```python
from build123d import *

# Parameters (mm, degrees)
SKETCH_1_R              = 12.5
EXTRUDE_1_DEPTH         = 111
SKETCH_2_R              = 17.5
EXTRUDE_2_DEPTH         = 3
SKETCH_3_R              = 10
EXTRUDE_3_DEPTH         = 8
CUT_EXTRUDE_1_DEPTH     = 4
HOLE_WIZARD_M8_1_D      = 6.8
HOLE_WIZARD_M8_1_DEPTH  = 23.75
HOLE_WIZARD_M8_1_TIP    = 2.042926105
HOLE_WIZARD_M12_1_D     = 10.2
HOLE_WIZARD_M12_1_DEPTH = 30.25
HOLE_WIZARD_M12_1_TIP   = 3.064389157
CHAMFER_1_SIZE          = 0.5


with BuildPart() as part:
    # 草图1 → 凸台-拉伸1 (new body)
    with BuildSketch(Plane.XY):
        Circle(SKETCH_1_R)
    extrude(amount=EXTRUDE_1_DEPTH)

    # 草图2 → 凸台-拉伸2 (add)
    with BuildSketch(Plane.XY.offset(111)):
        Circle(SKETCH_2_R)
    extrude(amount=EXTRUDE_2_DEPTH)

    # 草图3 → 凸台-拉伸3 (add)
    with BuildSketch(Plane.XY.offset(114)):
        Circle(SKETCH_3_R)
    extrude(amount=EXTRUDE_3_DEPTH)

    # 草图4 → 切除-拉伸1 (cut)
    with BuildSketch(Plane(origin=(0, 12.5, 0), x_dir=(1, 0, 0), z_dir=(0, 1, 0))):
        with BuildLine():
            Line((4, -10), (4, -102))
            ThreePointArc((4, -102), (0, -106), (-4, -102))
            Line((-4, -102), (-4, -10))
            ThreePointArc((-4, -10), (0, -6), (4, -10))
        make_face()
    extrude(amount=-CUT_EXTRUDE_1_DEPTH, mode=Mode.SUBTRACT)

    # M8 螺纹孔1
    with Locations(Plane.XY.offset(122)):
        with Locations((0, 0)):
            Hole(HOLE_WIZARD_M8_1_D / 2, depth=HOLE_WIZARD_M8_1_DEPTH)
            with Locations((0, 0, -(HOLE_WIZARD_M8_1_DEPTH + HOLE_WIZARD_M8_1_TIP / 2))):  # 118° drill point
                Cone(0, HOLE_WIZARD_M8_1_D / 2, HOLE_WIZARD_M8_1_TIP, mode=Mode.SUBTRACT)

    # M12 螺纹孔1
    with Locations(Plane(origin=(0, 0, 0), x_dir=(-1, 0, 0), z_dir=(0, 0, -1))):
        with Locations((0, 0)):
            Hole(HOLE_WIZARD_M12_1_D / 2, depth=HOLE_WIZARD_M12_1_DEPTH)
            with Locations((0, 0, -(HOLE_WIZARD_M12_1_DEPTH + HOLE_WIZARD_M12_1_TIP / 2))):  # 118° drill point
                Cone(0, HOLE_WIZARD_M12_1_D / 2, HOLE_WIZARD_M12_1_TIP, mode=Mode.SUBTRACT)

    # 倒角1
    chamfer_1_edges = [part.edges().sort_by_distance(p)[0] for p in [
        (-12.5, 0, 0),
    ]]
    chamfer(chamfer_1_edges, length=CHAMFER_1_SIZE)


solid = part.part
```
Part model, mm, in its own coordinate system. A direction names the side the tool comes from. Round coordinates to 2 decimals unless told otherwise and drop trailing zeros. Order: outer loops, then holes, each group sorted by start corner. A loop starts at its lowest first (then second) coordinate and runs counter-clockwise, first axis right, second up. Notation, with made-up numbers: M 48,7.5 L 91,7.5 A24 ccw 91,21.5 Z; hole C 25.5,-14.75 d9. An arc over 180 degrees is marked long. Answer in a Markdown table with one row per item. Add a question column.
Q1. Wall check: L1, parallel to Y at x = 0, z = 108; L2, parallel to Y at x = 0, z = 15.5; L3, parallel to Z at x = 13, y = 6.5. Give the ranges that are in metal, low to high. Write a range as from..to.
Q2. Cut at A-A on z = 58.5. Give the cut face in (x, y), and give its area (3 significant figures).
Q3. Mould opens along Y. For faces 1 (the face through (8, -11, 111)), 2 (the face through (0.192, -0.865, 32.782)), 3 (the face through (-2.17, -9.76, 117.94)) say: +Y half, -Y half, draft (parallel to the pull), parting line (faces both ways), or undercut.
Q4. Pin check, flat tips, straight feed: pin 1 (1.5 mm diameter, centred on y = 5.5, z = 104.5, fed in from -X); pin 2 (6 mm diameter, centred on y = -10, z = 82.5, fed in from -X); pin 3 (3.5 mm diameter, centred on y = 10.5, z = 71, fed in from -X). Stop position of each tip, or through.
Q5. 3-axis set-ups, long thin cutter, end or side, ignore diameter. For faces 4 (the face through (0, 11, 6)), 5 (the face through (0.74, -3.32, 109.96)), 6 (the face through (0, -4, 122)), 7 (the face through (5.77, -11.09, 54.98)), 8 (the face through (-13.887, -10.648, 112.479)): which of +Z, -Z, +X, -X, +Y, -Y reach the whole face in a straight line?
Established:
| question | item | result |
|---|---|---|
| 1 | L1 | y = -12.5..-3.4, 3.4..12.5 |
| 1 | L2 | y = -12.5..-5.1, 5.1..8.5 |
| 1 | L3 | z = 111..114 |
| 2 | outline | M -4,8.5 L -4,11.84 A12.5 ccw long 4,11.84 L 4,8.5 Z |
| 2 | area | 461 mm2 |
| 3 | face 1 | draft |
| 3 | face 2 | undercut |
| 3 | face 3 | parting line |
| 4 | pin 1 | stops at x = -11.56 |
| 4 | pin 2 | stops at x = -10.36 |
| 4 | pin 3 | stops at x = -8.93 |
| 5 | face 4 | +Y |
| 5 | face 5 | +Z |
| 5 | face 6 | +Z, +X, -X, +Y, -Y |
| 5 | face 7 | -Z |
| 5 | face 8 | +Z, -Z |
